The model under review builds one solid part; all positions refer to its coordinate system, in mm. A direction names the side the tool comes from. Coordinates: 2 decimals unless noted, no trailing zeros. Write each loop counter-clockwise with the first axis right and the second up, starting at its lowest first coordinate (ties: lowest second). Pieces come first, ordered by that corner, then holes. Notation, with made-up numbers: (-38.75, 5) - (1.25, 5) arc R19 cw to (1.25, 17) - close; hole circle Ø9 at (-10, 58.5). An arc over 180 degrees is marked (long way). Return JSON: item names as keys, results as strings. Group by question number.
(1) We need section C-C on y = -44. State the section outline as (x, z) points.
(2) We need section A-A on y = 24. State the section outline as (x, z) points, then the cut area to 3 significant figures.
(3) To check wall thickness, follow L1, parallel to Z at x = -34, y = -30; L2, parallel to Z at x = -23.5, y = -3.5; L3, parallel to Z at x = -12, y = -64.5. State the ranges of each line that lie inside material, in increasing order. Write a range as from..to.
(4) Tool access review of faces 4 (the face through (-4.686, 35.694, -79.734)), 5 (the face through (14, 36, 15)), 6 (the face through (-1, 1, 53)): name each direction out of +Z, -Z, +X, -X, +Y, -Y from which nothing blocks a thin tool from reaching the whole face with its end or side.
(5) For pin 1 Ø6 at (y, z) = (27, 27) entering from +X; pin 2 Ø3 at (x, z) = (27, 21.5) entering from -Y; pin 3 Ø3 at (y, z) = (12.5, 36) entering from +X, all flat-tipped, find the tip position at first contact; note any pin that passes through.
(6) Draft analysis for pull direction Z (two halves, no side actions). For faces 1 (the face through (14.515, -66.767, -22.678)), 2 (the face through (1.101, 79.992, -53.395)), 3 (the face through (-1, 1, -99)), state which applies: released by +Z, released by -Z, zero draft, split by the parting line, or undercut.
(7) We need section B-B on x = 53.5. State the section outline as (y, z) points.
(8) We need section D-D on z = -25. State the section outline as (x, y) points, then the cut area to 3 significant figures.
```python
from build123d import *

# Parameters (mm, degrees)
CRANK_WEB_DEPTH        = 15
CRANKPIN_PROFILE_R     = 27
CRANKPIN_DEPTH         = 46
MAIN_JOURNAL_PROFILE_R = 36
MAIN_JOURNAL_DEPTH     = 38


with BuildPart() as part:
    # Crank Web Profile → Crank Web (new body)
    with BuildSketch(Plane.XY):
        with BuildLine():
            ThreePointArc((66.583317356, 44.347061344), (0, 80), (-66.583317356, 44.347061344))
            Line((-66.583317356, 44.347061344), (-37.153763851, -55.005446241))
            ThreePointArc((-37.153763851, -55.005446241), (0, -82.749477613), (37.153763851, -55.005446241))
            Line((37.153763851, -55.005446241), (66.583317356, 44.347061344))
        make_face()
    crank_web = extrude(amount=CRANK_WEB_DEPTH)

    # Crankpin Profile → Crankpin (add)
    with BuildSketch(Plane(origin=(0, 0, 0), x_dir=(-1, 0, 0), z_dir=(0, 0, -1))):
        with Locations(Location((0, -44, 0), (0, 0, 180))):
            Circle(CRANKPIN_PROFILE_R)
    extrude(amount=CRANKPIN_DEPTH)

    # Main Journal Profile → Main Journal (add)
    with BuildSketch(Plane.XY.offset(15)):
        Circle(MAIN_JOURNAL_PROFILE_R)
    main_journal = extrude(amount=MAIN_JOURNAL_DEPTH)

    # Mirrored Web and Journal: Crank Web, Main Journal across plane
    add(crank_web.mirror(Plane(origin=(0, 0, -23), x_dir=(1, 0, 0), z_dir=(0, 0, -1))))
    add(main_journal.mirror(Plane(origin=(0, 0, -23), x_dir=(1, 0, 0), z_dir=(0, 0, -1))))


solid = part.part
```
Ans:
{
 "1": {"outline": "(-40.41, -61) - (40.41, -61) - (40.41, -46) - (27, -46) - (27, 0) - (40.41, 0) - (40.41, 15) - (-40.41, 15) - (-40.41, 0) - (-27, 0) - (-27, -46) - (-40.41, -46) - close"},
 "2": {"outline": "(-60.56, -61) - (-26.83, -61) - (-26.83, -99) - (26.83, -99) - (26.83, -61) - (60.56, -61) - (60.56, -46) - (-60.56, -46) - close; (-60.56, 0) - (60.56, 0) - (60.56, 15) - (26.83, 15) - (26.83, 53) - (-26.83, 53) - (-26.83, 15) - (-60.56, 15) - close", "area": "7,710 mm²"},
 "3": {"L1": "-61..-46, 0..15", "L2": "-99..-46, 0..53", "L3": "-61..15"},
 "4": {"face 4": "-Z", "face 5": "+Z", "face 6": "+Z, +X, -X, +Y, -Y"},
 "5": {"pin 1": "x = 26.83", "pin 2": "y = -25.41", "pin 3": "x = 34.28"},
 "6": {"face 1": "undercut", "face 2": "zero draft", "face 3": "released by -Z"},
 "7": {"outline": "(0.18, -61) - (59.48, -61) - (59.48, -46) - (0.18, -46) - close; (0.18, 0) - (59.48, 0) - (59.48, 15) - (0.18, 15) - close"},
 "8": {"outline": "circle Ø54 at (0, -44)", "area": "2,290 mm²"}
}
